from build123d import *

# Parameters (mm, degrees)
SKETCH1_R           = 6.1
BOSS_EXTRUDE1_DEPTH = 10
BOSS_EXTRUDE2_DEPTH = 2.5
SKETCH3_R           = 2
CUT_EXTRUDE1_DEPTH  = 22.729473072
SKETCH4_R           = 5.6
CUT_EXTRUDE2_DEPTH  = 5
CHAMFER1_SIZE       = 0.72


with BuildPart() as part:
    # Sketch1 → Boss-Extrude1 (new body)
    with BuildSketch(Plane(origin=(0, 0, 0), x_dir=(1, 0, 0), z_dir=(0, 1, 0))):
        with Locations(Location((0, 0, 0), (0, 0, 270))):
            Circle(SKETCH1_R)
    extrude(amount=BOSS_EXTRUDE1_DEPTH)

    # Sketch2 → Boss-Extrude2 (add, symmetric)
    with BuildSketch(Plane(origin=(0, 0, 0), x_dir=(0, 0, -1), z_dir=(1, 0, 0))):
        with BuildLine():
            Line((-4.992659986, 10), (-4.475823522, 14.965836668))
            ThreePointArc((-4.475823522, 14.965836668), (0, 19), (4.475823522, 14.965836668))
            Line((4.475823522, 14.965836668), (4.992659986, 10))
            Line((4.992659986, 10), (-4.992659986, 10))
        make_face()
    extrude(amount=BOSS_EXTRUDE2_DEPTH, both=True)

    # Sketch3 → Cut-Extrude1 (cut, through all)
    with BuildSketch(Plane(origin=(2.5, 0, 0), x_dir=(0, 0, -1), z_dir=(1, 0, 0))):
        with Locations((0, 16)):
            Circle(SKETCH3_R)
    extrude(amount=-CUT_EXTRUDE1_DEPTH, mode=Mode.SUBTRACT)

    # Sketch4 → Cut-Extrude2 (cut)
    with BuildSketch(Plane.XZ):
        with Locations(Location((0, 0, 0), (0, 0, 270))):
            Circle(SKETCH4_R)
    extrude(amount=-CUT_EXTRUDE2_DEPTH, mode=Mode.SUBTRACT)

    # Chamfer1
    chamfer1_edges = [part.edges().sort_by_distance(p)[0] for p in [
        (0, 5, 5.6),
    ]]
    chamfer(chamfer1_edges, length=CHAMFER1_SIZE)


solid = part.part
Could you check a few things on this model? Use its own coordinates, in mm. A direction names the side the tool comes from. Give positions to 0.01 mm unless a question says otherwise; leave off trailing zeros. Order: outer loops, then holes, each group sorted by start corner. A loop starts at its lowest first (then second) coordinate and runs counter-clockwise, first axis right, second up. Notation, with made-up numbers: (87.25, 74) - (105.25, 74) arc R6 cw to (105.25, 81) - close; hole circle Ø3 at (2, 56). An arc over 180 degrees is marked (long way). One line per item, written item: value. Start each with the question number.
1. Imagine slicing it at C-C on y = 16. List the corners of the cut face in (x, z) for me, plus the area to 3 significant figures.
2. Thinking about a two-plate mould opening in Z: for faces 6 (the face through (0.035, 12.448, 4.738)), 7 (the face through (0.246, 2.11, 5.595)), 8 (the face through (0, 19, 0)), which applies, +Z half, -Z half, draft (parallel to the pull), parting line (faces both ways), or undercut?
3. If I drill on probe 1 along X at (y, z) = (1.9, 0); probe 2 along Y at (x, z) = (1.1, 0); probe 3 along X at (y, z) = (13.5, 0), over which ranges is the centre line in solid material (lowest first)?
4. Imagine slicing it at D-D on y = 7.5. List the corners of the cut face in (x, z) for me, plus the area to 3 significant figures.
5. For P1, Ø5, axis at x = -5, y = 9, coming from the -Z side; P2, Ø5, axis at x = -0.5, z = 1.5, coming from the -Y side; P3, Ø3, axis at y = 16, z = -3.5, coming from the +X side; P4, Ø3, axis at y = 16, z = 0, coming from the -X side, each with a flat end and sliding along its axis, tell me the tip position at first contact or that it passes through.
6. For faces 1 (the face through (2.5, 13.6, -0.1)), 2 (the face through (0, 5, 0)), 3 (the face through (-2.5, 13.6, -0.1)), 4 (the face through (0.04, 12.52, -4.73)), 5 (the face through (-5, 0, 3)), which set-ups out of +Z, -Z, +X, -X, +Y, -Y let a thin tool reach every point of the face, with its end or its side?
7. Imagine slicing it at B-B on x = 0. List the corners of the cut face in (y, z) for me, plus the area to 3 significant figures.
8. Imagine slicing it at A-A on z = 0. List the corners of the cut face in (x, y) for me, plus the area to 3 significant figures.
Values:
1. outline: (-2.5, -4.24) - (2.5, -4.24) - (2.5, -2) - (-2.5, -2) - close; (-2.5, 2) - (2.5, 2) - (2.5, 4.24) - (-2.5, 4.24) - close
1. area: 22.4 mm²
2. face 6: +Z half
2. face 7: undercut
2. face 8: parting line
3. probe 1: -6.1 to -5.6, 5.6 to 6.1
3. probe 2: 5 to 14, 18 to 19
3. probe 3: -2.5 to 2.5
4. outline: circle Ø12.2 at (0, 0)
4. area: 117 mm²
5. P1: z = -5.56
5. P2: y = 5
5. P3: x = 2.5
5. P4: through
6. face 1: +Z, -Z, +X, +Y
6. face 2: -Y
6. face 3: +Z, -Z, -X, +Y
6. face 4: -Z, +X, -X, +Y
6. face 5: +Z, -Z, +X, -X, -Y
7. outline: (0, -6.1) - (10, -6.1) - (10, -4.99) - (14.97, -4.48) arc R4.5 ccw to (14.97, 4.48) - (10, 4.99) - (10, 6.1) - (0, 6.1) - (0, 5.6) - (4.28, 5.6) - (5, 4.88) - (5, -4.88) - (4.28, -5.6) - (0, -5.6) - close; hole circle Ø4 at (16, 0)
7. area: 129 mm²
8. outline: (-6.1, 0) - (-5.6, 0) - (-5.6, 4.28) - (-4.88, 5) - (4.88, 5) - (5.6, 4.28) - (5.6, 0) - (6.1, 0) - (6.1, 10) - (2.5, 10) - (2.5, 14) - (-2.5, 14) - (-2.5, 10) - (-6.1, 10) - close; (-2.5, 18) - (2.5, 18) - (2.5, 19) - (-2.5, 19) - close
8. area: 91.5 mm²
